For this review, use the dimensioned drawing (mm, ordinates from the lowest corner) and the shaded views. A direction names the side the tool comes from. Give positions to 0.01 mm unless a question says otherwise; leave off trailing zeros. Loops run counter-clockwise (first coordinate to the right, second up) from the corner with the lowest first, then second, coordinate; pieces in that order, holes last. Notation, with made-up numbers: (32, 8) -> (46, 8) arc R23 cw to (46, 44) -> close; hole circle Ø7 at (73, 63.5). An arc over 180 degrees is marked (long way). Write each question's results on one line, items separated by ' | '. Start each with the question number.
Q1. Machinability: for the marked faces 4 and 5, which of the approach directions +Z, -Z, +X, -X, +Y, -Y give a long, thin tool a straight path to every point of the face, cutting with its end or side? Answer none if there is none.
Q2. Wall thickness on L1, parallel to Y at x = 5, z = 11.5; L2, parallel to X at y = 2.25, z = 8; L3, parallel to Y at x = 5, z = 22.3: over which ranges is each line inside the solid? List them lowest first. Write a range as [from, to].
Q3. We need section A-A (y = 5). Write out the cut boundary in (x, z).
Q4. Insertion check: pin 1 Ø4 at (x, y) = (4, 6) entering from -Z; pin 2 Ø1 at (x, y) = (10.5, 7.5) entering from -Z. Each pin has a flat end and moves straight along its axis. Give the tip position at first contact, or say it passes through.
Q5. We need section B-B (x = 5). Write out the cut boundary in (y, z), plus the area to 3 significant figures.
Q6. We need section D-D (z = 17.5). Write out the cut boundary in (x, y).
Q7. We need section C-C (z = 12.5). Write out the cut boundary in (x, y), plus the area to 3 significant figures.
Q8. Mouldability with a two-part tool opening along X and no side actions: class the marked faces 1, 2 and 3 as released by +X, released by -X, zero draft, split by the parting line, or undercut.
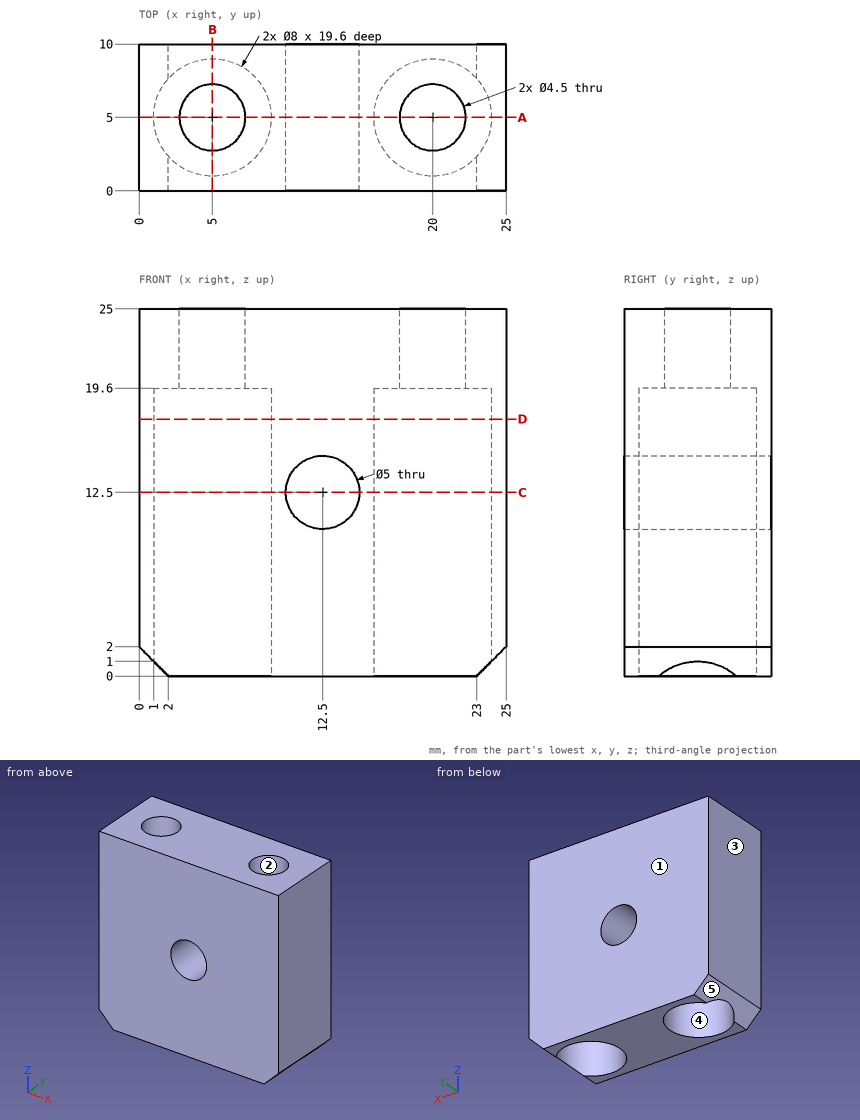
Output:
1) face 4: -Z | face 5: -Z, -X, +Y, -Y
2) L1: [0, 1], [9, 10] | L2: [0, 2.1], [7.9, 17.1], [22.9, 25] | L3: [0, 2.75], [7.25, 10]
3) outline: (0, 2) -> (1, 1) -> (1, 19.6) -> (2.75, 19.6) -> (2.75, 25) -> (0, 25) -> close; (7.25, 19.6) -> (9, 19.6) -> (9, 0) -> (16, 0) -> (16, 19.6) -> (17.75, 19.6) -> (17.75, 25) -> (7.25, 25) -> close; (22.25, 19.6) -> (24, 19.6) -> (24, 1) -> (25, 2) -> (25, 25) -> (22.25, 25) -> close; hole circle Ø5 at (12.5, 12.5)
4) pin 1: z = 19.6 | pin 2: z = 0
5) outline: (0, 0) -> (1, 0) -> (1, 19.6) -> (2.75, 19.6) -> (2.75, 25) -> (0, 25) -> close; (7.25, 19.6) -> (9, 19.6) -> (9, 0) -> (10, 0) -> (10, 25) -> (7.25, 25) -> close | area: 68.9 mm2
6) outline: (0, 0) -> (25, 0) -> (25, 10) -> (0, 10) -> close; hole circle Ø8 at (5, 5); hole circle Ø8 at (20, 5)
7) outline: (0, 0) -> (10, 0) -> (10, 10) -> (0, 10) -> close; (15, 0) -> (25, 0) -> (25, 10) -> (15, 10) -> close; hole circle Ø8 at (5, 5); hole circle Ø8 at (20, 5) | area: 99.5 mm2
8) face 1: zero draft | face 2: undercut | face 3: released by -X
